```python
from build123d import *

# Parameters (mm, degrees)
SKETCH_1_W          = 200
SKETCH_1_H          = 310
EXTRUDE_1_DEPTH     = 5
SKETCH_2_W          = 100
SKETCH_2_H          = 50
CUT_EXTRUDE_1_DEPTH = 185.729532019
HOLE_WIZARD_M5_2_D  = 4.2
FILLET_1_R          = 10
HOLE_WIZARD_M5_4_D  = 4.2
HOLE_WIZARD_M5_5_D  = 4.2
HOLE_WIZARD_M5_6_D  = 4.2


with BuildPart() as part:
    # 草图1 → 凸台-拉伸1 (new, symmetric)
    with BuildSketch(Plane.XY):
        Rectangle(SKETCH_1_W, SKETCH_1_H)
    extrude(amount=EXTRUDE_1_DEPTH, both=True)

    # 草图2 → 切除-拉伸1 (cut, through all)
    with BuildSketch(Plane.XY.offset(5)):
        with Locations((0, -105)):
            Rectangle(SKETCH_2_W, SKETCH_2_H)
    extrude(amount=-CUT_EXTRUDE_1_DEPTH, mode=Mode.SUBTRACT)

    # M5 螺纹孔2 (through all)
    with Locations(Plane.XY.offset(5)):
        with Locations((85, -130), (85, -30), (-85, -30), (-85, -130)):
            Hole(HOLE_WIZARD_M5_2_D / 2)

    # 圆角1
    fillet_1_edges = [part.edges().sort_by_distance(p)[0] for p in [
        (50, -80, 0),
        (50, -130, 0),
        (-50, -130, 0),
        (-50, -80, 0),
    ]]
    fillet(fillet_1_edges, radius=FILLET_1_R)

    # M5 螺纹孔4 (through all)
    with Locations(Plane(origin=(0, 0, -5), x_dir=(-1, 0, 0), z_dir=(0, 0, -1))):
        with Locations((92.5, 120), (92.5, 140), (-92.5, 140), (-92.5, 120)):
            Hole(HOLE_WIZARD_M5_4_D / 2)

    # M5 螺纹孔5 (through all)
    with Locations(Plane(origin=(0, 0, -5), x_dir=(-1, 0, 0), z_dir=(0, 0, -1))):
        with Locations((-57.5, -105), (57.5, -105)):
            Hole(HOLE_WIZARD_M5_5_D / 2)

    # M5 螺纹孔6 (through all)
    with Locations(Plane(origin=(0, 0, -5), x_dir=(-1, 0, 0), z_dir=(0, 0, -1))):
        with Locations((90, -143.5), (90, -103.5), (-90, -103.5), (-90, -143.5)):
            Hole(HOLE_WIZARD_M5_6_D / 2)


solid = part.part
```
The listing builds one solid part. Answer for the finished solid, in the listing's coordinates (mm). A direction names the side the tool comes from. Give positions to 0.01 mm unless a question says otherwise; leave off trailing zeros. Loops run counter-clockwise (first coordinate to the right, second up) from the corner with the lowest first, then second, coordinate; pieces in that order, holes last. Notation, with made-up numbers: M 79,29.25 L 83,29.25 A34 ccw 83,67.25 Z; hole C 49,-28.5 d10. An arc over 180 degrees is marked long. One line per item, written item: value.
Q1. Determine the mould class of faces 3 (the face through (-47.15, -83.01, -0.07)), 4 (the face through (-1, 2, 5)), 5 (the face through (-100, -2, 0)) for opening direction X: +X half, -X half, draft (parallel to the pull), parting line (faces both ways), or undercut.
Working result:
face 3: undercut
face 4: draft
face 5: -X half
Q2. Find the intervals of material crossed by line 1 (Y direction, x = -85, z = -3); line 2 (Y direction, x = -92.5, z = -0.25); line 3 (X direction, y = 140, z = -1), in increasing order. Write a range as from..to.
Working result:
line 1: y = -155..-132.1, -127.9..-32.1, -27.9..155
line 2: y = -155..117.9, 122.1..137.9, 142.1..155
line 3: x = -100..-94.6, -90.4..90.4, 94.6..100
Q3. A cutting plane is placed at B-B on x = 3. Determine the outline of the cut face in (y, z), then the cut area to 3 significant figures.
Working result:
outline: M -155,-5 L -130,-5 L -130,5 L -155,5 Z; M -80,-5 L 155,-5 L 155,5 L -80,5 Z
area: 2,600 mm^2
Q4. For faces 1 (the face through (-46.99, -127.15, -0.07)), 2 (the face through (-1, 155, 0)), determine the directions among +Z, -Z, +X, -X, +Y, -Y from which every point of the face is accessible in a straight line to the end or side of a thin tool.
Working result:
face 1: +Z, -Z
face 2: +Z, -Z, +X, -X, +Y
Q5. A cutting plane is placed at A-A on z = -2.5. Give the number of separate pieces and of enclosed holes in the cut face, then the cut area to 3 significant figures.
Working result:
separate pieces: 1
enclosed holes: 15
area: 56,900 mm^2
